```python
from build123d import *

# Parameters (mm, degrees)
SKETCH_1_W          = 494.5
SKETCH_1_H          = 1168
SKETCH_1_R          = 3.25
EXTRUDE_1_DEPTH     = 2
SKETCH_2_W          = 2.5
SKETCH_2_H          = 2
CUT_EXTRUDE_1_DEPTH = 1194.884652092


with BuildPart() as part:
    # 草图1 → 凸台-拉伸1 (new body)
    with BuildSketch(Plane.XY):
        Rectangle(SKETCH_1_W, SKETCH_1_H)
        with Locations((-237.25, 0)):
            Circle(SKETCH_1_R, mode=Mode.SUBTRACT)
        with Locations((-237.25, -126)):
            Circle(SKETCH_1_R, mode=Mode.SUBTRACT)
        with Locations((-237.25, -252)):
            Circle(SKETCH_1_R, mode=Mode.SUBTRACT)
        with Locations((-237.25, -378)):
            Circle(SKETCH_1_R, mode=Mode.SUBTRACT)
        with Locations((-237.25, -504)):
            Circle(SKETCH_1_R, mode=Mode.SUBTRACT)
        with Locations((0, -574)):
            Circle(SKETCH_1_R, mode=Mode.SUBTRACT)
        with Locations(Location((0, 574, 0), (0, 0, 180))):
            Circle(SKETCH_1_R, mode=Mode.SUBTRACT)
        with Locations(Location((-237.25, 504, 0), (0, 0, 180))):
            Circle(SKETCH_1_R, mode=Mode.SUBTRACT)
        with Locations(Location((-237.25, 378, 0), (0, 0, 180))):
            Circle(SKETCH_1_R, mode=Mode.SUBTRACT)
        with Locations(Location((-237.25, 252, 0), (0, 0, 180))):
            Circle(SKETCH_1_R, mode=Mode.SUBTRACT)
        with Locations(Location((-237.25, 126, 0), (0, 0, 180))):
            Circle(SKETCH_1_R, mode=Mode.SUBTRACT)
        with Locations((237.25, 126)):
            Circle(SKETCH_1_R, mode=Mode.SUBTRACT)
        with Locations((237.25, 252)):
            Circle(SKETCH_1_R, mode=Mode.SUBTRACT)
        with Locations((237.25, 378)):
            Circle(SKETCH_1_R, mode=Mode.SUBTRACT)
        with Locations((237.25, 504)):
            Circle(SKETCH_1_R, mode=Mode.SUBTRACT)
        with Locations(Location((237.25, -504, 0), (0, 0, 180))):
            Circle(SKETCH_1_R, mode=Mode.SUBTRACT)
        with Locations(Location((237.25, -378, 0), (0, 0, 180))):
            Circle(SKETCH_1_R, mode=Mode.SUBTRACT)
        with Locations(Location((237.25, -252, 0), (0, 0, 180))):
            Circle(SKETCH_1_R, mode=Mode.SUBTRACT)
        with Locations(Location((237.25, -126, 0), (0, 0, 180))):
            Circle(SKETCH_1_R, mode=Mode.SUBTRACT)
        with Locations(Location((237.25, 0, 0), (0, 0, 180))):
            Circle(SKETCH_1_R, mode=Mode.SUBTRACT)
        with Locations((-210, 574)):
            Circle(SKETCH_1_R, mode=Mode.SUBTRACT)
        with Locations((210, 574)):
            Circle(SKETCH_1_R, mode=Mode.SUBTRACT)
        with Locations(Location((-210, -574, 0), (0, 0, 180))):
            Circle(SKETCH_1_R, mode=Mode.SUBTRACT)
        with Locations(Location((210, -574, 0), (0, 0, 180))):
            Circle(SKETCH_1_R, mode=Mode.SUBTRACT)
    extrude(amount=EXTRUDE_1_DEPTH)

    # 草图2 → 切除-拉伸1 (cut, through all)
    with BuildSketch(Plane.XZ.offset(584)):
        with Locations((246, 1)):
            Rectangle(SKETCH_2_W, SKETCH_2_H)
    extrude(amount=-CUT_EXTRUDE_1_DEPTH, mode=Mode.SUBTRACT)


solid = part.part
```
The listing builds one solid part. Answer for the finished solid, in the listing's coordinates (mm). Coordinates: 2 decimals unless noted, no trailing zeros. Answer as a JSON object with one key per item and string values. Group by question number.
1. Straight lines are drawn through the part: line 1 (X direction, y = 574, z = 1.5); line 2 (X direction, y = -381, z = 1.3). For each, find the intervals that lie inside material, in ascending order.
2. A flat-ended cylindrical pin translates along its axis: P1, Ø6, axis at x = -237.25, y = 504, coming from the -Z side. Find the tip coordinate at first contact, or state that the pin passes through.
3. Determine the mould class of faces 1 (the flat face through (-5, 8, 2)), 2 (the flat face through (-5, 8, 0)) for opening direction Z: released by +Z, released by -Z, zero draft, split by the parting line, or undercut.
Values follow:
{
 "1": {"line 1": "-247.25 to -213.25, -206.75 to -3.25, 3.25 to 206.75, 213.25 to 244.75", "line 2": "-247.25 to -238.5, -236 to 236, 238.5 to 244.75"},
 "2": {"P1": "through"},
 "3": {"face 1": "released by +Z", "face 2": "released by -Z"}
}
